Answer from the drawing. Dimensions are ordinates in mm from the lowest x, y and z of the part. Coordinates: 2 decimals unless noted, no trailing zeros. Write each loop counter-clockwise with the first axis right and the second up, starting at its lowest first coordinate (ties: lowest second). Pieces come first, ordered by that corner, then holes. Notation, with made-up numbers: (85, -38) - (89, -38) arc R33 ccw to (89, -3) - close; hole circle Ø9 at (1.25, -20). An arc over 180 degrees is marked (long way). Return JSON: item names as keys, results as strings.
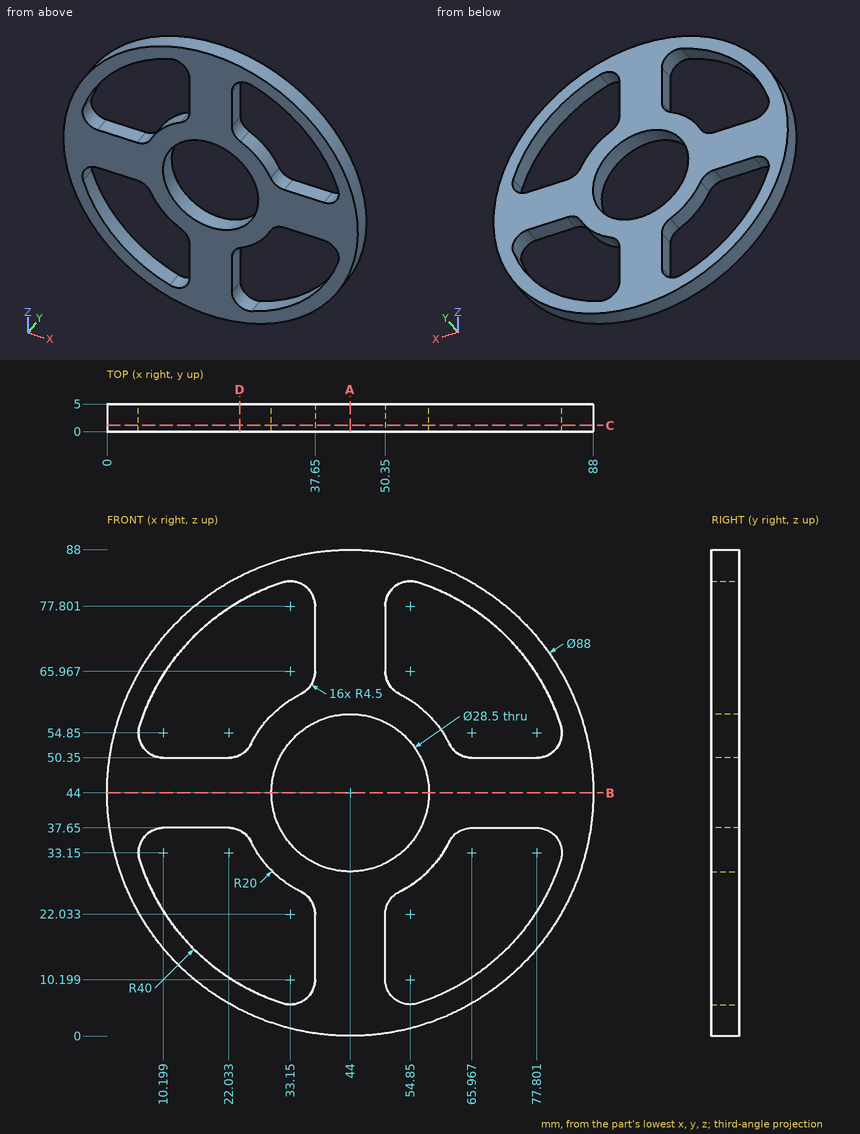
(1) A cutting plane is placed at A-A (x = 44). Determine the outline of the cut face in (y, z).
Answer:
{"outline": "(0, 0) - (5, 0) - (5, 29.75) - (0, 29.75) - close; (0, 58.25) - (5, 58.25) - (5, 88) - (0, 88) - close"}
(2) A cutting plane is placed at B-B (z = 44). Determine the outline of the cut face in (x, y).
Answer:
{"outline": "(0, 0) - (29.75, 0) - (29.75, 5) - (0, 5) - close; (58.25, 0) - (88, 0) - (88, 5) - (58.25, 5) - close"}
(3) A cutting plane is placed at D-D (x = 24). Determine the outline of the cut face in (y, z).
Answer:
{"outline": "(0, 4.81) - (5, 4.81) - (5, 9.36) - (0, 9.36) - close; (0, 37.2) - (5, 37.2) - (5, 50.8) - (0, 50.8) - close; (0, 78.64) - (5, 78.64) - (5, 83.19) - (0, 83.19) - close"}
(4) Straight lines are drawn through the part: line 1 (Z direction, x = 19.5, y = 3.65); line 2 (X direction, y = 3.55, z = 27) (1 decimal); line 3 (X direction, y = 0.75, z = 56.5) (1 decimal). For each, find the intervals that lie inside material, in ascending order. Write a range as from..to.
Answer:
{"line 1": "7.45..12.38, 37.65..50.35, 75.62..80.55", "line 2": "3.4..7.8, 33.5..54.5, 80.2..84.6", "line 3": "1.8..6, 28.4..37.2, 50.8..59.6, 82..86.2"}
(5) A cutting plane is placed at C-C (y = 1.15). State how many separate pieces and enclosed holes the cut face has, and give its area (3 significant figures).
Answer:
{"separate pieces": "1", "enclosed holes": "5", "area": "2,770 mm²"}
(6) Flat-ended cylindrical pins translate along their axes: P1, Ø1.5, axis at y = 2, z = 14, coming from the +X side; P2, Ø2.5, axis at x = 15, y = 2.5, coming from the -Z side (1 decimal); P3, Ø2.5, axis at x = 13.5, y = 2.5, coming from the +Z side. Find the tip coordinate at first contact, or state that the pin passes through.
Answer:
{"P1": "x = 76.87", "P2": "z = 9.9", "P3": "z = 76.87"}
